Source: CAD feature listing. Evaluate the final solid. Frame: model axes, mm. Face numbers are marked on the shaded views. A direction names the side the tool comes from. Give positions to 0.01 mm unless a question says otherwise; leave off trailing zeros. Order: outer loops, then holes, each group sorted by start corner. A loop starts at its lowest first (then second) coordinate and runs counter-clockwise, first axis right, second up. Notation, with made-up numbers: (65.5, -10) -> (122.5, -10) arc R22 cw to (122.5, 26) -> close; hole circle Ø3 at (38.25, 50.25). An arc over 180 degrees is marked (long way). Use CSV: the item, a comma, the result in double quotes.
```python
from build123d import *

# Parameters (mm, degrees)
SHAFT_PROFILE_12_R   = 6
SHAFT_12_DEPTH       = 30
COLLAR_PROFILE_19_R  = 9.5
COLLAR_19_DEPTH      = 25
CROSS_HOLE_PROFILE_R = 2
CROSS_HOLE_DEPTH     = 12.5


with BuildPart() as part:
    # Shaft Profile Ø12 → Shaft Ø12 (new body)
    with BuildSketch(Plane(origin=(0, 0, 0), x_dir=(1, 0, 0), z_dir=(0, 1, 0))):
        with Locations(Location((0, 0, 0), (0, 0, 270))):
            Circle(SHAFT_PROFILE_12_R)
    extrude(amount=SHAFT_12_DEPTH)

    # Collar Profile Ø19 → Collar Ø19 (add)
    with BuildSketch(Plane(origin=(0, 30, 0), x_dir=(1, 0, 0), z_dir=(0, 1, 0))):
        with Locations(Location((0, 0, 0), (0, 0, 270))):
            Circle(COLLAR_PROFILE_19_R)
    extrude(amount=COLLAR_19_DEPTH)

    # Dome Head Profile → Dome Head (revolve)
    with BuildSketch(Plane(origin=(0, 0, 0), x_dir=(0, 0, -1), z_dir=(1, 0, 0))):
        with BuildLine():
            Line((0, 55), (-19, 55))
            ThreePointArc((-19, 55), (-10.604187915, 61.769260733), (0, 63.734903146))
            Line((0, 63.734903146), (0, 55))
        make_face()
    revolve(axis=Axis((0, 55, 0), (0, 1, 0)))

    # Cross Hole Profile → Cross Hole (cut, symmetric)
    with BuildSketch(Plane(origin=(0, 0, 0), x_dir=(0, 0, -1), z_dir=(1, 0, 0))):
        with Locations((0, 8)):
            Circle(CROSS_HOLE_PROFILE_R)
    extrude(amount=CROSS_HOLE_DEPTH, both=True, mode=Mode.SUBTRACT)


solid = part.part
```
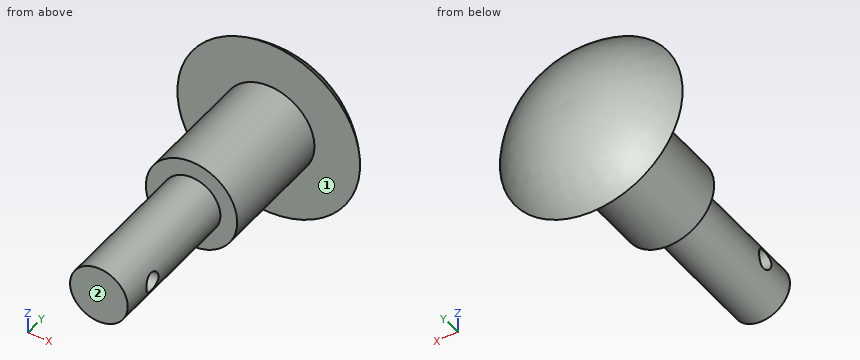
1. Section query B-B on y = 8. Return loops of the section in (x, z), plus the area to 3 significant figures.
Answer below:
outline,"(-5.66, -2) arc R6 ccw to (5.66, -2) -> close; (-5.66, 2) -> (5.66, 2) arc R6 ccw to start"
area,"66.0 mm²"
2. Section query A-A on y = 41.5. Return loops of the section in (x, z), plus the area to 3 significant figures.
Answer below:
outline,"circle Ø19 at (0, 0)"
area,"284 mm²"
3. Ray query, line 1 along Z through (x, y) = (-2, 9.5); line 2 along Z through (x, y) = (-2, 8); line 3 along Y through (x, z) = (4, 0.5). Return the intervals inside material, ascending.
Answer below:
line 1,"z = -5.66 to -1.32, 1.32 to 5.66"
line 2,"z = -5.66 to -2, 2 to 5.66"
line 3,"y = 0 to 6.06, 9.94 to 63.62"
4. Pin query (flat end, axial travel): P1, Ø3, axis at x = 11, z = 9.5, coming from the -Y side; P2, Ø12, axis at y = 12.5, z = 13.5, coming from the -X side; P3, Ø1.5, axis at y = 38, z = -8, coming from the +X side; P4, Ø6, axis at y = 33, z = 5, coming from the +X side. Return the tip coordinate at first contact, or that it passes through.
Answer below:
P1,"stops at y = 55"
P2,"passes through"
P3,"stops at x = 6.14"
P4,"stops at x = 9.29"
5. Access query for the marked faces 1 and 2. Directions: +Z, -Z, +X, -X, +Y, -Y. A direction counts if a zero-diameter tool reaches every point of the face in a straight line with its end or side. Return the directions, or none.
Answer below:
face 1,"-Y"
face 2,"+Z, -Z, +X, -X, -Y"
